```python
from build123d import *

# Parameters (mm, degrees)
SKETCH1_W           = 180
SKETCH1_H           = 50
BOSS_EXTRUDE1_DEPTH = 40
SKETCH2_W           = 113.5
SKETCH2_H           = 20.5
CUT_EXTRUDE1_DEPTH  = 102.612007165
SKETCH3_R           = 1.5
CUT_EXTRUDE2_DEPTH  = 102.612007165
SKETCH4_W           = 101.523941395
SKETCH4_H           = 14
CUT_EXTRUDE3_DEPTH  = 30
SKETCH5_W           = 113.5
SKETCH5_H           = 14.75
CUT_EXTRUDE4_DEPTH  = 14
CHAMFER1_SIZE       = 10


with BuildPart() as part:
    # Sketch1 → Boss-Extrude1 (new body)
    with BuildSketch(Plane.XY):
        Rectangle(SKETCH1_W, SKETCH1_H)
    extrude(amount=BOSS_EXTRUDE1_DEPTH)

    # Sketch2 → Cut-Extrude1 (cut, through all)
    with BuildSketch(Plane.XY.offset(40)):
        Rectangle(SKETCH2_W, SKETCH2_H)
    extrude(amount=-CUT_EXTRUDE1_DEPTH, mode=Mode.SUBTRACT)

    # Sketch3 → Cut-Extrude2 (cut, through all)
    with BuildSketch(Plane.XY.offset(40)):
        with Locations((-56.75, 10.25)):
            Circle(SKETCH3_R)
        with Locations((-56.75, -10.25)):
            Circle(SKETCH3_R)
        with Locations((56.75, 10.25)):
            Circle(SKETCH3_R)
        with Locations((56.75, -10.25)):
            Circle(SKETCH3_R)
    extrude(amount=-CUT_EXTRUDE2_DEPTH, mode=Mode.SUBTRACT)

    # Sketch4 → Cut-Extrude3 (cut)
    with BuildSketch(Plane(origin=(0, 25, 0), x_dir=(1, 0, 0), z_dir=(0, 1, 0))):
        with Locations((-0.398466407, -7)):
            Rectangle(SKETCH4_W, SKETCH4_H)
    extrude(amount=-CUT_EXTRUDE3_DEPTH, mode=Mode.SUBTRACT)

    # Sketch5 → Cut-Extrude4 (cut)
    with BuildSketch(Plane(origin=(0, 0, 0), x_dir=(-1, 0, 0), z_dir=(0, 0, -1))):
        with Locations((0, -17.625)):
            Rectangle(SKETCH5_W, SKETCH5_H)
    extrude(amount=-CUT_EXTRUDE4_DEPTH, mode=Mode.SUBTRACT)

    # Chamfer1
    chamfer1_edges = [part.edges().sort_by_distance(p)[0] for p in [
        (90, 0, 40),
        (-90, 0, 40),
    ]]
    chamfer(chamfer1_edges, length=CHAMFER1_SIZE)


solid = part.part
```
Geometry check sheet. Reference: the model listing, model coordinates, mm. A direction names the side the tool comes from. Coordinates: 2 decimals unless noted, no trailing zeros. Write each loop counter-clockwise with the first axis right and the second up, starting at its lowest first coordinate (ties: lowest second). Pieces come first, ordered by that corner, then holes. Notation, with made-up numbers: M 64.5,-20 L 74.5,-20 A29 ccw 74.5,2 Z; hole C -6.75,8.5 d5. An arc over 180 degrees is marked long. Use one line per item in the form item = value. Start each with the question number.
1) Section check D-D on z = 33. Enter the section's corners in (x, y).
2) Go/stop test with flat-tipped pins: pin 1 Ø10 at (y, z) = (-17, 34.5) entering from +X; pin 2 Ø7.5 at (x, y) = (0.5, -20.5) entering from -Z; pin 3 Ø2.5 at (x, y) = (56.75, -10.25) entering from +Z. Record where each tip stops, or that it passes through.
3) Thickness scan on probe 1 along X at (y, z) = (-10.25, 11.5); probe 2 along Y at (x, z) = (20.5, 34); probe 3 along X at (y, z) = (-14, 8.5). Record the ranges inside material, lowest first. Write a range as from..to.
4) Section check B-B on z = 3. Enter the section's corners in (x, y), and give its area (3 significant figures).
5) Set-up check for faces 4 (the flat face through (-56.75, -18, 7)), 5 (the flat face through (-1, 10.25, 29)), 6 (the flat face through (-51.16, 18, 7)), 7 (the flat face through (-85, 0, 35)): record each of +Z, -Z, +X, -X, +Y, -Y from which the full face is reachable in a straight line by a thin tool's end or side.
6) Section check C-C on y = -3. Enter the section's corners in (x, z).
7) Section check A-A on x = 7.5. Enter the section's corners in (y, z), and give its area (3 significant figures).
8) Release check for a two-part mould opening along Y. For faces 1 (the flat face through (-1, 25, 24)), 2 (the cylindrical face through (-57.775, 11.345, 20.28)), 3 (the flat face through (1, -18, 14)) record: pulls with the +Y half, pulls with the -Y half, needs draft (parallel to the pull), parting line crosses it, or undercut.
Responses:
q1.outline = M -87,-25 L 87,-25 L 87,25 L -87,25 Z; hole M -56.75,-8.75 A1.5 ccw long -55.25,-10.25 L 55.25,-10.25 A1.5 ccw long 56.75,-8.75 L 56.75,8.75 A1.5 ccw long 55.25,10.25 L -55.25,10.25 A1.5 ccw long -56.75,8.75 Z
q2.pin_1 = 90
q2.pin_2 = 14
q2.pin_3 = through
q3.probe_1 = -90..-58.25, 58.25..90
q3.probe_2 = -25..-10.25, 10.25..25
q3.probe_3 = -90..-56.75, 56.75..90
q4.outline = M -90,-25 L -56.75,-25 L -56.75,-11.75 A1.5 cw -56.75,-8.75 L -56.75,8.75 A1.5 cw long -55.25,10.25 L -51.16,10.25 L -51.16,25 L -90,25 Z; M 50.36,10.25 L 55.25,10.25 A1.5 cw long 56.75,8.75 L 56.75,-8.75 A1.5 cw 56.75,-11.75 L 56.75,-25 L 90,-25 L 90,25 L 50.36,25 Z
q4.area = 3,480 mm2
q5.face_4 = -Z, -Y
q5.face_5 = +Z, -Z
q5.face_6 = -Z, +Y, -Y
q5.face_7 = +Z, -X, +Y, -Y
q6.outline = M -90,0 L -56.75,0 L -56.75,40 L -80,40 L -90,30 Z; M 56.75,0 L 90,0 L 90,30 L 80,40 L 56.75,40 Z
q7.outline = M -25,14 L -10.25,14 L -10.25,40 L -25,40 Z; M 10.25,14 L 25,14 L 25,40 L 10.25,40 Z
q7.area = 767 mm2
q8.face_1 = pulls with the +Y half
q8.face_2 = undercut
q8.face_3 = needs draft
